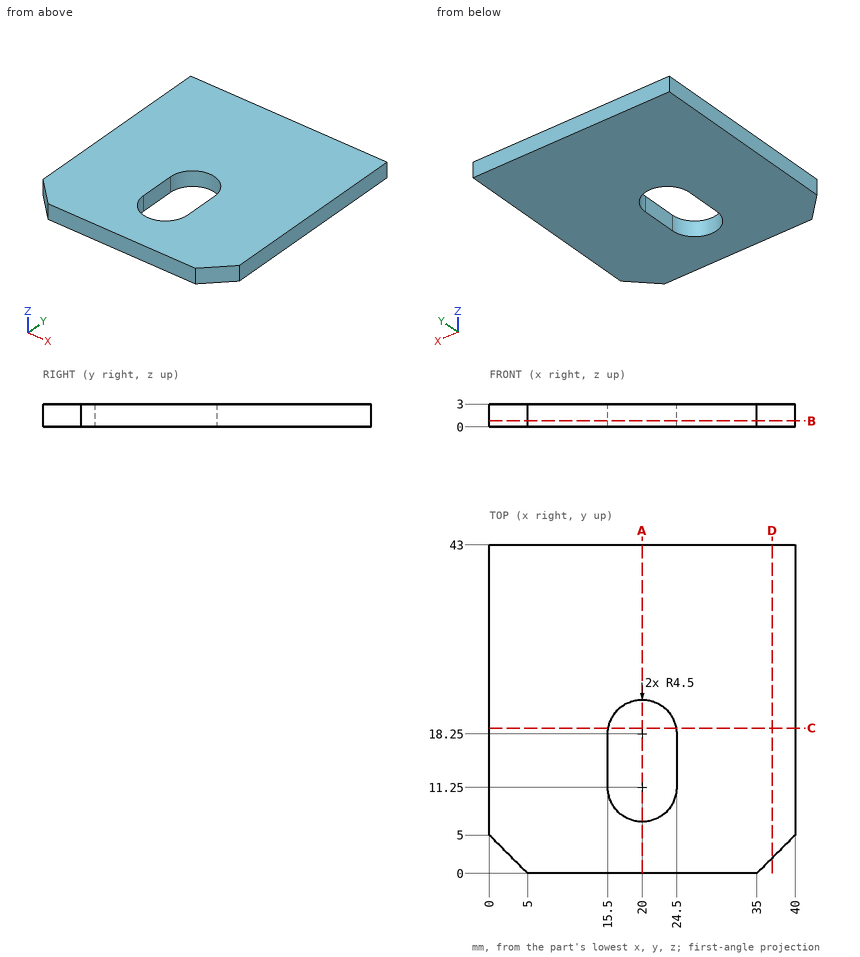
Check sheet for the drawn part. Datum: minimum x, y, z corner. Units: mm. Round coordinates to 2 decimals unless told otherwise and drop trailing zeros. Loops run counter-clockwise (first coordinate to the right, second up) from the corner with the lowest first, then second, coordinate; pieces in that order, holes last. Notation, with made-up numbers: M 18.5,10 L 42.5,10 A22 cw 42.5,43 Z; hole C 72,-28 d7. An arc over 180 degrees is marked long. One line per question, with ' | ' between items. Start each with the question number.
Item 1: Scan lines: probe 1 along X at (y, z) = (12, 2.35); probe 2 along Y at (x, z) = (16, 0.9); probe 3 along Y at (x, z) = (22, 1.2). Record each from-to range of solid material in increasing order.
Item 2: Section check D-D (x = 37). Record the boundary of the cut face in (y, z).
Item 3: Section check C-C (y = 19). Record the boundary of the cut face in (x, z), and give its area (3 significant figures).
Item 4: Section check B-B (z = 0.8). Record the boundary of the cut face in (x, y), and give its area (3 significant figures).
Item 5: Section check A-A (x = 20). Record the boundary of the cut face in (y, z).
Worked out:
1) probe 1: 0 to 15.5, 24.5 to 40 | probe 2: 0 to 9.19, 20.31 to 43 | probe 3: 0 to 7.22, 22.28 to 43
2) outline: M 2,0 L 43,0 L 43,3 L 2,3 Z
3) outline: M 0,0 L 15.56,0 L 15.56,3 L 0,3 Z; M 24.44,0 L 40,0 L 40,3 L 24.44,3 Z | area: 93.4 mm^2
4) outline: M 0,5 L 5,0 L 35,0 L 40,5 L 40,43 L 0,43 Z; hole M 15.5,11.25 A4.5 ccw 24.5,11.25 L 24.5,18.25 A4.5 ccw 15.5,18.25 Z | area: 1,570 mm^2
5) outline: M 0,0 L 6.75,0 L 6.75,3 L 0,3 Z; M 22.75,0 L 43,0 L 43,3 L 22.75,3 Z
